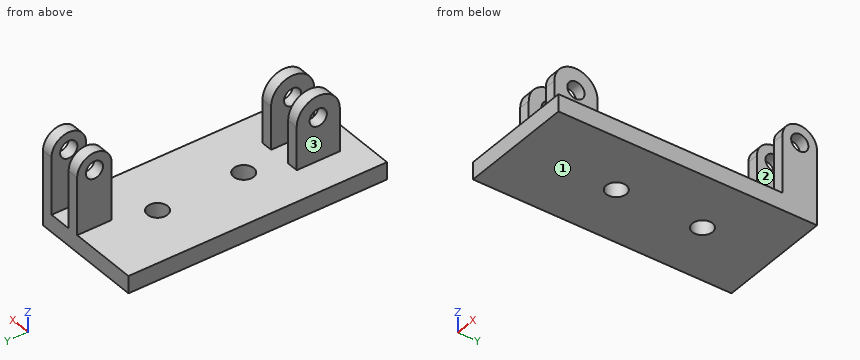
from build123d import *

# Parameters (mm, degrees)
SKETCH1_W           = 40
SKETCH1_H           = 90
BOSS_EXTRUDE1_DEPTH = 6
SKETCH3_R           = 3
BOSS_EXTRUDE2_DEPTH = 4
BOSS_EXTRUDE3_START = 4
SKETCH4_R           = 3
BOSS_EXTRUDE3_DEPTH = 4
LPATTERN1_COUNT     = 2
LPATTERN1_PITCH     = 12
SKETCH5_R           = 3.5
CUT_EXTRUDE1_DEPTH  = 56.686623169


with BuildPart() as part:
    # Sketch1 → Boss-Extrude1 (new body)
    with BuildSketch(Plane.XY):
        Rectangle(SKETCH1_W, SKETCH1_H)
    extrude(amount=BOSS_EXTRUDE1_DEPTH)

    # Sketch3 → Boss-Extrude2 (add)
    with BuildSketch(Plane.ZY.offset(-20)):
        with BuildLine():
            Line((26, 45), (6, 45))
            Line((6, 45), (6, 33))
            Line((6, 33), (26, 33))
            ThreePointArc((26, 33), (32, 39), (26, 45))
        make_face()
        with Locations(Location((26, 39, 0), (0, 0, 270))):
            Circle(SKETCH3_R, mode=Mode.SUBTRACT)
    boss_extrude2 = extrude(amount=BOSS_EXTRUDE2_DEPTH)

    # Sketch4 → Boss-Extrude3 (add)
    with BuildSketch(Plane(origin=(0, 0, 0), x_dir=(0, 0, -1), z_dir=(1, 0, 0)).offset(BOSS_EXTRUDE3_START)):
        with BuildLine():
            Line((-21, -22.5), (-6, -22.5))
            Line((-6, -22.5), (-6, -37.5))
            Line((-6, -37.5), (-21, -37.5))
            ThreePointArc((-21, -37.5), (-28.5, -30), (-21, -22.5))
        make_face()
        with Locations((-21, -30)):
            Circle(SKETCH4_R, mode=Mode.SUBTRACT)
    boss_extrude3 = extrude(amount=BOSS_EXTRUDE3_DEPTH)

    # Mirror1: Boss-Extrude3 across plane
    add(boss_extrude3.mirror(Plane(origin=(0, 0, 0), x_dir=(0, 0, 1), z_dir=(1, 0, 0))))

    # LPattern1: Boss-Extrude2 ×2
    with Locations(*[(-i * LPATTERN1_PITCH, 0, 0) for i in range(1, LPATTERN1_COUNT)]):
        add(boss_extrude2)

    # Sketch5 → Cut-Extrude1 (cut, through all)
    with BuildSketch(Plane.XY.offset(6)):
        with Locations((0, 20)):
            Circle(SKETCH5_R)
        with Locations((0, -10)):
            Circle(SKETCH5_R)
    extrude(amount=-CUT_EXTRUDE1_DEPTH, mode=Mode.SUBTRACT)


solid = part.part
CAD build for the part. Positions are in the model's coordinates, mm. Face numbers are marked on the shaded views. A direction names the side the tool comes from. Round coordinates to 2 decimals unless told otherwise and drop trailing zeros. Loops run counter-clockwise (first coordinate to the right, second up) from the corner with the lowest first, then second, coordinate; pieces in that order, holes last. Notation, with made-up numbers: M 11.25,52.5 L 31.25,52.5 A22 ccw 31.25,66.5 Z; hole C 72,-28.75 d6. An arc over 180 degrees is marked long. One line per question, with ' | ' between items. Start each with the question number.
Item 1: Wall check: line 1 (Y direction, x = 0, z = 4); line 2 (Y direction, x = 4.9, z = 21); line 3 (X direction, y = -34.5, z = 25.5). Give the ranges that are in metal, low to high.
Item 2: Which spindle directions (+Z, -Z, +X, -X, +Y, -Y) get a long thin tool onto all of the face, cutting with end or side? Do the marked faces 1, 2 and 3. Say none if no direction does.
Item 3: Cut at C-C, the plane y = 20. Write the cut outline in (x, z), plus the area to 3 significant figures.
Item 4: Cut at B-B, the plane x = 0. Write the cut outline in (y, z), plus the area to 3 significant figures.
Item 5: Pin check, flat tips, straight feed: pin 1 Ø3.5 at (y, z) = (41.5, 18.5) entering from -X; pin 2 Ø4.5 at (x, z) = (-6.5, 11.5) entering from -Y; pin 3 Ø10 at (x, z) = (14, 24) entering from -Y; pin 4 Ø3.5 at (y, z) = (39, 26) entering from +X. Stop position of each tip, or through.
Item 6: Cut at A-A, the plane y = 39. Write the cut outline in (x, z), plus the area to 3 significant figures.
Item 7: Cut at D-D, the plane x = 7. Write the cut outline in (y, z), plus the area to 3 significant figures.
Responses:
1) line 1: y = -45 to -13.5, -6.5 to 16.5, 23.5 to 45 | line 2: y = -37.5 to -33, -27 to -22.5, 33 to 45 | line 3: x = -8 to -4, 4 to 8
2) face 1: -Z, +X, -X, +Y, -Y | face 2: +Z, +Y, -Y | face 3: +Z, -X, +Y, -Y
3) outline: M -20,0 L -3.5,0 L -3.5,6 L -20,6 Z; M 3.5,0 L 20,0 L 20,6 L 3.5,6 Z | area: 198 mm²
4) outline: M -45,0 L -13.5,0 L -13.5,6 L -45,6 Z; M -6.5,0 L 16.5,0 L 16.5,6 L -6.5,6 Z; M 23.5,0 L 45,0 L 45,6 L 23.5,6 Z | area: 456 mm²
5) pin 1: stops at x = 4 | pin 2: stops at y = -37.5 | pin 3: stops at y = 33 | pin 4: passes through
6) outline: M -20,0 L 20,0 L 20,23 L 16,23 L 16,6 L 8,6 L 8,23 L 4,23 L 4,6 L -20,6 Z; M 4,29 L 8,29 L 8,32 L 4,32 Z; M 16,29 L 20,29 L 20,32 L 16,32 Z | area: 400 mm²
7) outline: M -45,0 L 45,0 L 45,26 A6 ccw 33,26 L 33,6 L -22.5,6 L -22.5,21 A7.5 ccw -37.5,21 L -37.5,6 L -45,6 Z; hole C -30,21 d6; hole C 39,26 d6 | area: 1,090 mm²
